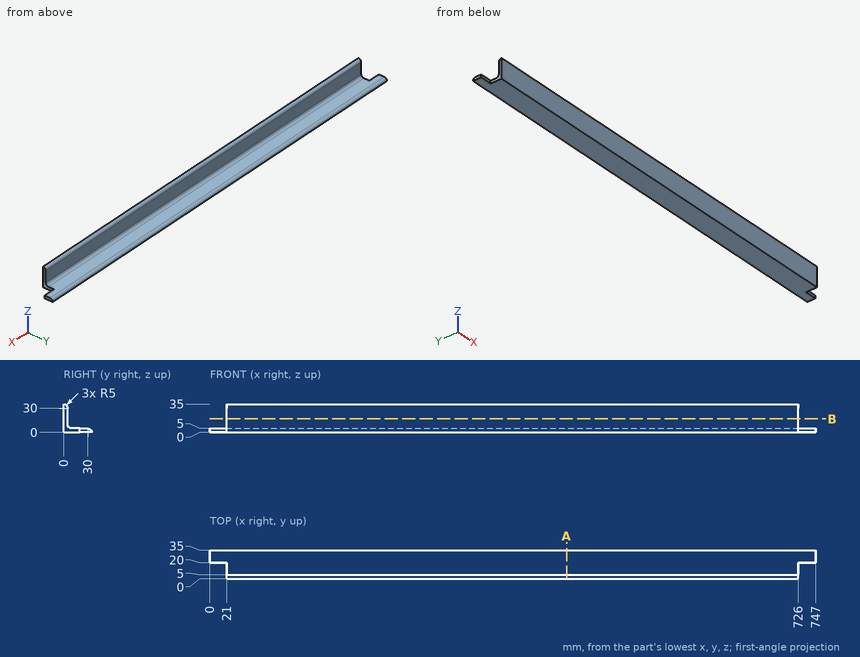
Geometry check sheet. Reference: drawing and pictorial views, mm from the part's lowest x, y, z. Coordinates: 2 decimals unless noted, no trailing zeros. Order: outer loops, then holes, each group sorted by start corner. A loop starts at its lowest first (then second) coordinate and runs counter-clockwise, first axis right, second up. Notation, with made-up numbers: M -3.5,59 L 9.5,59 A7 ccw 9.5,68 Z; hole C -35.75,-4 d6. An arc over 180 degrees is marked long. Return JSON: item names as keys, results as strings.
1) Cross-section at A-A, the plane x = 440. Record the boundary of the cut face in (y, z).
Answer list:
{"outline": "M 0,0 L 35,0 A5 ccw 30,5 L 10,5 A5 cw 5,10 L 5,30 A5 ccw 0,35 Z"}
2) Thickness scan on L1, parallel to Z at x = 342, y = 22; L2, parallel to X at y = 2, z = 29. Record the ranges inside material, lowest first. Write a range as [from, to].
Answer list:
{"L1": "[0, 5]", "L2": "[21, 726]"}
3) Cross-section at B-B, the plane z = 16.5. Record the boundary of the cut face in (x, y), and give its area (4 significant figures).
Answer list:
{"outline": "M 21,0 L 726,0 L 726,5 L 21,5 Z", "area": "3,525 mm2"}
4) Gauge pin test, flat ends, axial feed: pin 1 (1.5 mm diameter, centred on x = 735, z = 2.5, fed in from -Y); pin 2 (2 mm diameter, centred on x = 264, z = 15.5, fed in from +Y); pin 3 (16 mm diameter, centred on y = 8, z = 25, fed in from -X); pin 4 (16 mm diameter, centred on y = 14, z = 25, fed in from +X). Record the tip position at first contact, or that the pin passes through.
Answer list:
{"pin 1": "y = 20", "pin 2": "y = 5", "pin 3": "x = 21", "pin 4": "through"}
